Could you check a few things on this model? Use its own coordinates, in mm. A direction names the side the tool comes from. Coordinates: 2 decimals unless noted, no trailing zeros. Loops run counter-clockwise (first coordinate to the right, second up) from the corner with the lowest first, then second, coordinate; pieces in that order, holes last. Notation, with made-up numbers: (-9, 74) - (3, 74) arc R13 cw to (3, 91) - close; hole circle Ø8 at (49.5, 18). An arc over 180 degrees is marked (long way). Put each result on its own line as item: value. Start each with the question number.
```python
from build123d import *

# Parameters (mm, degrees)
SKETCH_1_W          = 4.25
SKETCH_1_H          = 5
SKETCH_2_R          = 2.5
EXTRUDE_1_DEPTH     = 16
CUT_EXTRUDE_1_DEPTH = 2.5
CHAMFER_1_SIZE      = 0.425


with BuildPart() as part:
    # 草图1 → 旋转1 (revolve)
    with BuildSketch(Plane(origin=(0, 0, 0), x_dir=(1, 0, 0), z_dir=(0, 1, 0))):
        with Locations((2.125, -2.5)):
            Rectangle(SKETCH_1_W, SKETCH_1_H)
    revolve(axis=Axis((0, 0, 0), (0, 0, 1)))

    # 草图2 → 凸台-拉伸1 (add)
    with BuildSketch(Plane(origin=(0, 0, 0), x_dir=(-1, 0, 0), z_dir=(0, 0, -1))):
        Circle(SKETCH_2_R)
    extrude(amount=EXTRUDE_1_DEPTH)

    # 草图3 → 切除-拉伸1 (cut)
    with BuildSketch(Plane.XY.offset(5)):
        Polygon((2, 1.154700538), (0, 2.309401077), (-2, 1.154700538), (-2, -1.154700538), (0, -2.309401077), (2, -1.154700538), align=None)
    extrude(amount=-CUT_EXTRUDE_1_DEPTH, mode=Mode.SUBTRACT)

    # 草图4 → 切除-旋转1 (revolve, cut)
    with BuildSketch(Plane.XZ, mode=Mode.PRIVATE) as cut_revolve_1_sk:
        Polygon((2, 2.5), (0, 2.5), (0, 1.345299462), align=None)
    revolve(cut_revolve_1_sk.sketch.rotate(Axis((0, 0, 2.5), (0, 0, -1)), 90), axis=Axis((0, 0, 2.5), (0, 0, -1)), mode=Mode.SUBTRACT)

    # 倒角1
    chamfer_1_edges = [part.edges().sort_by_distance(p)[0] for p in [
        (-4.25, 0, 5),
        (2.5, 0, -16),
    ]]
    chamfer(chamfer_1_edges, length=CHAMFER_1_SIZE)


solid = part.part
```
(1) I need wall thicknesses on L1, parallel to Z at x = -2.75, y = 2; L2, parallel to X at y = -1.5, z = -13; L3, parallel to Y at x = 0, z = -9. Which ranges of each line are inside material? Lowest first, please. Write a range as [from, to].
(2) I want a section at B-B on z = -4.5. List the corners of the cut face in (x, y) for me.
(3) If we mould it in two halves opening along X, with no side actions, what happens to faces 3 (the flat face through (0.99, -1.74, 3.77)), 4 (the cylindrical face through (0.54, -2.44, -7.68)), 5 (the flat face through (-2, -2, 0))? For each: pulls with the +X half, pulls with the -X half, needs draft (parallel to the pull), parting line crosses it, or undercut.
(4) For pin 1 Ø2 at (y, z) = (-2, -10) entering from -X; pin 2 Ø5 at (y, z) = (0.5, -11.5) entering from +X; pin 3 Ø4 at (x, z) = (1.5, -9) entering from -Y, each with a flat end and sliding along its axis, tell me the tip position at first contact or that it passes through.
(5) I want a section at A-A on z = 2.25. List the corners of the cut face in (x, y) for me.
(6) Which directions (+Z, -Z, +X, -X, +Y, -Y) give clear straight access to the entire face, cutting with the end or side of a thin tool? Please do faces 1 (the flat face through (0, 0, -16)), 2 (the flat face through (1.014, 1.724, 3.768)).
Answer sheet:
1. L1: z = [0, 5]
1. L2: x = [-2, 2]
1. L3: y = [-2.5, 2.5]
2. outline: circle Ø5 at (0, 0)
3. face 3: undercut
3. face 4: parting line crosses it
3. face 5: needs draft
4. pin 1: stops at x = -2.29
4. pin 2: stops at x = 2.5
4. pin 3: stops at y = -2.5
5. outline: circle Ø8.5 at (0, 0); hole circle Ø3.13 at (0, 0)
6. face 1: -Z, +X, -X, +Y, -Y
6. face 2: +Z
